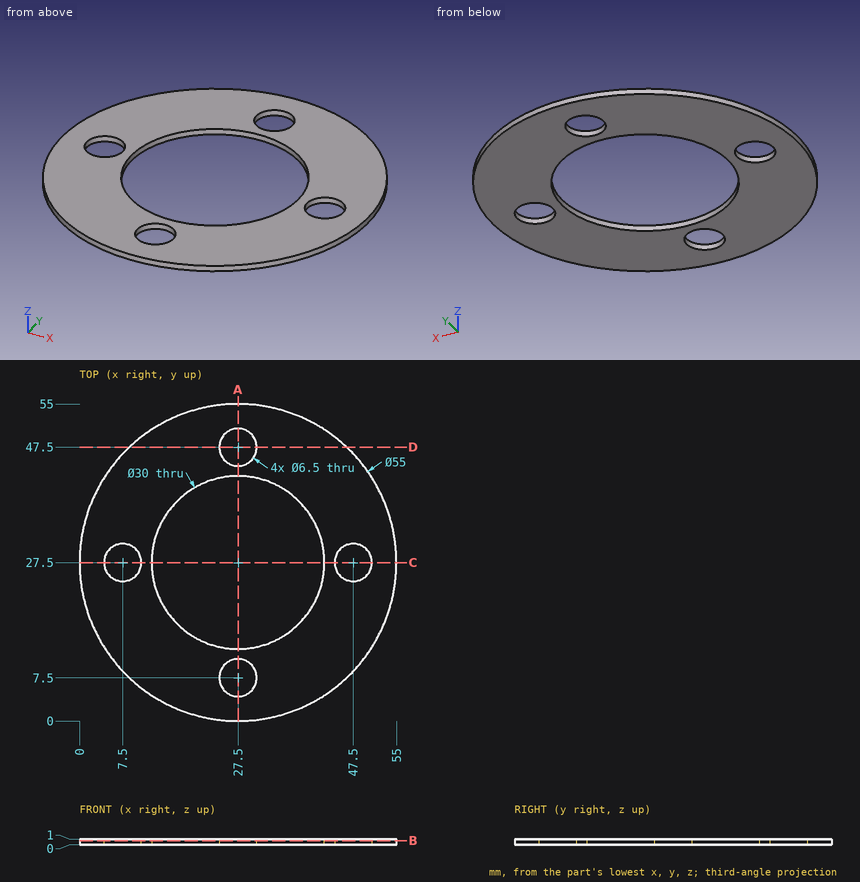
The drawing under review shows one solid part. Ordinate dimensions are in mm from its lowest x, y, z. Round coordinates to 2 decimals unless told otherwise and drop trailing zeros. Write each loop counter-clockwise with the first axis right and the second up, starting at its lowest first coordinate (ties: lowest second). Pieces come first, ordered by that corner, then holes. Notation, with made-up numbers: (-12.75, 28.5) - (17.25, 28.5) arc R17 cw to (17.25, 46.5) - close; hole circle Ø3 at (4, -24.75). An arc over 180 degrees is marked (long way). Use a Markdown table: item, result. Add a question column.
1. We need section D-D (y = 47.5). State the section outline as (x, z) points, then the cut area to 3 significant figures.
2. We need section B-B (z = 0.7). State the section outline as (x, y) points.
3. We need section A-A (x = 27.5). State the section outline as (y, z) points, then the cut area to 3 significant figures.
4. Wall thickness on probe 1 along Y at (x, z) = (27.5, 0.8); probe 2 along Y at (x, z) = (19.5, 0.2); probe 3 along Y at (x, z) = (10.5, 0.75): over which ranges is each line inside the solid? List them lowest first.
5. Clearance check with flat-ended pins moving along their axes: pin 1 (5 mm diameter, centred on x = 40.5, y = 34, fed in from +Z); pin 2 (24 mm diameter, centred on x = 27.5, y = 27.5, fed in from -Z) (3 decimals). State where each tip first meets the part, or that it passes through.
Output:
| question | item | result |
|---|---|---|
| 1 | outline | (8.63, 0) - (24.25, 0) - (24.25, 1) - (8.63, 1) - close; (30.75, 0) - (46.37, 0) - (46.37, 1) - (30.75, 1) - close |
| 1 | area | 31.2 mm2 |
| 2 | outline | circle Ø55 at (27.5, 27.5); hole circle Ø6.5 at (7.5, 27.5); hole circle Ø30 at (27.5, 27.5); hole circle Ø6.5 at (27.5, 7.5); hole circle Ø6.5 at (27.5, 47.5); hole circle Ø6.5 at (47.5, 27.5) |
| 3 | outline | (0, 0) - (4.25, 0) - (4.25, 1) - (0, 1) - close; (10.75, 0) - (12.5, 0) - (12.5, 1) - (10.75, 1) - close; (42.5, 0) - (44.25, 0) - (44.25, 1) - (42.5, 1) - close; (50.75, 0) - (55, 0) - (55, 1) - (50.75, 1) - close |
| 3 | area | 12.0 mm2 |
| 4 | probe 1 | y = 0 to 4.25, 10.75 to 12.5, 42.5 to 44.25, 50.75 to 55 |
| 4 | probe 2 | y = 1.19 to 14.81, 40.19 to 53.81 |
| 4 | probe 3 | y = 5.88 to 26.25, 28.75 to 49.12 |
| 5 | pin 1 | stops at z = 1 |
| 5 | pin 2 | passes through |
